The listing builds one solid part. Answer for the finished solid, in the listing's coordinates (mm). A direction names the side the tool comes from. Round coordinates to 2 decimals unless told otherwise and drop trailing zeros. Write each loop counter-clockwise with the first axis right and the second up, starting at its lowest first coordinate (ties: lowest second). Pieces come first, ordered by that corner, then holes. Notation, with made-up numbers: M 31.25,41.5 L 60.25,41.5 A16 ccw 60.25,59.5 Z; hole C -3.75,-5 d3. An arc over 180 degrees is marked long. Put each result on its own line as item: value. Start each with the question number.
```python
from build123d import *

# Parameters (mm, degrees)
SKETCH1_W                  = 80
SKETCH1_H                  = 16
BOSS_EXTRUDE1_DEPTH        = 20
SKETCH2_R                  = 5
CUT_EXTRUDE1_DEPTH         = 20
SKETCH4_R                  = 6
CUT_EXTRUDE2_DEPTH         = 16.5
SKETCH5_W                  = 29.106163607
SKETCH5_H                  = 1
SKETCH5_W_2                = 37.036491662
CUT_EXTRUDE3_DEPTH         = 30
M6_TAPPED_HOLE1_AT_2_COUNT = 2
M6_TAPPED_HOLE1_AT_2_PITCH = 68
SKETCH8_R                  = 3.25
CUT_EXTRUDE4_DEPTH         = 30
SKETCH9_R                  = 5
CUT_EXTRUDE5_DEPTH         = 4


with BuildPart() as part:
    # Sketch1 → Boss-Extrude1 (new body)
    with BuildSketch(Plane.XY):
        with Locations((9.337676654, 6.4605919)):
            Rectangle(SKETCH1_W, SKETCH1_H)
        with BuildLine():
            Line((-3.162323346, 11.7105919), (21.837676654, 11.7105919))
            ThreePointArc((21.837676654, 11.7105919), (27.087676654, 6.4605919), (21.837676654, 1.2105919))
            Line((21.837676654, 1.2105919), (-3.162323346, 1.2105919))
            ThreePointArc((-3.162323346, 1.2105919), (-8.412323346, 6.4605919), (-3.162323346, 11.7105919))
        make_face(mode=Mode.SUBTRACT)
    extrude(amount=BOSS_EXTRUDE1_DEPTH)

    # Sketch2 → Cut-Extrude1 (cut)
    with BuildSketch(Plane.XZ.offset(1.5394081)):
        with Locations(Location((34.337676654, 10, 0), (0, 0, 270))):
            Circle(SKETCH2_R)
        with Locations(Location((-15.662323346, 10, 0), (0, 0, 270))):
            Circle(SKETCH2_R)
    extrude(amount=-CUT_EXTRUDE1_DEPTH, mode=Mode.SUBTRACT)

    # Sketch4 → Cut-Extrude2 (cut, symmetric)
    with BuildSketch(Plane.XZ.offset(-11.7105919)):
        with Locations(Location((9.337676654, 10, 0), (0, 0, 270))):
            Circle(SKETCH4_R)
    extrude(amount=CUT_EXTRUDE2_DEPTH, both=True, mode=Mode.SUBTRACT)

    # Sketch5 → Cut-Extrude3 (cut)
    with BuildSketch(Plane.XZ.offset(1.5394081)):
        with Locations((48.890758457, 10)):
            Rectangle(SKETCH5_W, SKETCH5_H)
        with Locations((-34.180569177, 10)):
            Rectangle(SKETCH5_W_2, SKETCH5_H)
    extrude(amount=-CUT_EXTRUDE3_DEPTH, mode=Mode.SUBTRACT)

    # Sketch6 → M6 Tapped Hole1 (revolve, cut)
    with BuildSketch(Plane(origin=(43.337676654, 6.4605919, 9.5), x_dir=(0, -1, 0), z_dir=(1, 0, 0))):
        Polygon((0, 0), (0, 18.502151548), (2.5, 17), (2.5, 0), align=None)
    m6_tapped_hole1 = revolve(axis=Axis((43.337676654, 6.4605919, 15.85), (0, 0, -1)), mode=Mode.SUBTRACT)

    # M6 Tapped Hole1 at 2: M6 Tapped Hole1 ×2
    with Locations(*[(-i * M6_TAPPED_HOLE1_AT_2_PITCH, 0, 0) for i in range(1, M6_TAPPED_HOLE1_AT_2_COUNT)]):
        add(m6_tapped_hole1, mode=Mode.SUBTRACT)

    # Sketch8 → Cut-Extrude4 (cut)
    with BuildSketch(Plane(origin=(0, 0, 10.5), x_dir=(-1, 0, 0), z_dir=(0, 0, -1))):
        with Locations((24.662323346, 6.4605919)):
            Circle(SKETCH8_R)
        with Locations((-43.337676654, 6.4605919)):
            Circle(SKETCH8_R)
    extrude(amount=-CUT_EXTRUDE4_DEPTH, mode=Mode.SUBTRACT)

    # Sketch9 → Cut-Extrude5 (cut)
    with BuildSketch(Plane.XY.offset(20)):
        with Locations((43.337676654, 6.4605919)):
            Circle(SKETCH9_R)
        with Locations((-24.662323346, 6.4605919)):
            Circle(SKETCH9_R)
    extrude(amount=-CUT_EXTRUDE5_DEPTH, mode=Mode.SUBTRACT)


solid = part.part
```
Item 1: Section C-C (y = 10.75) is taken. Give the vertices of the cut face in (x, z), and give its area (3 significant figures).
Item 2: Flat-ended cylindrical pins translate along their axes: pin 1 (3 mm diameter, centred on x = 41, y = 7, fed in from +Z); pin 2 (6 mm diameter, centred on x = 43.34, y = 6.46, fed in from +Z). Find the tip coordinate at first contact, or state that the pin passes through.
Item 3: Consider line 1 along X through (y, z) = (12, 14); line 2 along Y through (x, z) = (2.5, 12); line 3 along X through (y, z) = (3.75, 17.25). Determine where each line is inside the solid, lowest interval first. Write a range as [from, to].
Item 4: Which of the six approach directions +Z, -Z, +X, -X, +Y, -Y give full straight-line access (tool end or side, diameter ignored) to faces 5 (the cylindrical face through (40.336, 5.216, 13.212)), 6 (the flat face through (46.5, 4.6, 10.5)), 7 (the flat face through (-27, 5, 9.5)), 8 (the cylindrical face through (-8.41, 6.35, 9.86))?
Item 5: Section D-D (x = 35) is taken. Give the vertices of the cut face in (y, z), and give its area (3 significant figures).
Item 6: Determine the mould class of faces 1 (the cylindrical face through (-10.667, 6.349, 9.787)), 2 (the flat face through (-28, 5, 10.5)), 3 (the flat face through (9, 14.461, 3)), 4 (the flat face through (-21, 7, 16)) for opening direction Z: released by +Z, released by -Z, zero draft, split by the parting line, or undercut.
Item 7: Section A-A (x = 17) is taken. Give the vertices of the cut face in (y, z), and give its area (3 significant figures).
Item 8: Section B-B (z = 6.5) is taken. Give the vertices of the cut face in (x, y), and give its area (3 significant figures).
Output values:
1. outline: M -30.66,0 L -6.19,0 L -6.19,20 L -22.09,20 L -22.09,16 L -27.23,16 L -27.23,20 L -30.66,20 L -30.66,10.5 L -20.64,10.5 A5 cw long -20.64,9.5 L -30.66,9.5 Z; M 24.86,0 L 49.34,0 L 49.34,9.5 L 39.31,9.5 A5 cw long 39.31,10.5 L 49.34,10.5 L 49.34,20 L 45.91,20 L 45.91,16 L 40.77,16 L 40.77,20 L 24.86,20 Z
1. area: 761 mm^2
2. pin 1: stops at z = 16
2. pin 2: stops at z = 9.5
3. line 1: x = [-30.66, -18.66], [-12.66, 4.87], [13.81, 31.34], [37.34, 49.34]
3. line 2: y = [-1.54, 1.21], [11.71, 14.46]
3. line 3: x = [-30.66, -28.86], [-20.46, -7.66], [26.33, 39.14], [47.54, 49.34]
4. face 5: +Z
4. face 6: +X, +Y, -Y
4. face 7: -X, +Y, -Y
4. face 8: +Z, -Z
5. outline: M -1.54,0 L 14.46,0 L 14.46,5.04 L -1.54,5.04 Z; M -1.54,14.96 L 14.46,14.96 L 14.46,20 L -1.54,20 Z
5. area: 161 mm^2
6. face 1: undercut
6. face 2: undercut
6. face 3: zero draft
6. face 4: released by +Z
7. outline: M -1.54,0 L 1.21,0 L 1.21,20 L -1.54,20 Z; M 11.71,0 L 14.46,0 L 14.46,20 L 11.71,20 Z
7. area: 110 mm^2
8. outline: M -30.66,-1.54 L -19.23,-1.54 L -19.23,14.46 L -30.66,14.46 Z; M -12.09,-1.54 L 4.46,-1.54 L 4.46,1.21 L -3.16,1.21 A5.25 cw -3.16,11.71 L 4.46,11.71 L 4.46,14.46 L -12.09,14.46 Z; M 14.21,-1.54 L 30.77,-1.54 L 30.77,14.46 L 14.21,14.46 L 14.21,11.71 L 21.84,11.71 A5.25 cw 21.84,1.21 L 14.21,1.21 Z; M 37.91,-1.54 L 49.34,-1.54 L 49.34,14.46 L 37.91,14.46 Z; hole C -24.66,6.46 d5; hole C 43.34,6.46 d5
8. area: 610 mm^2
